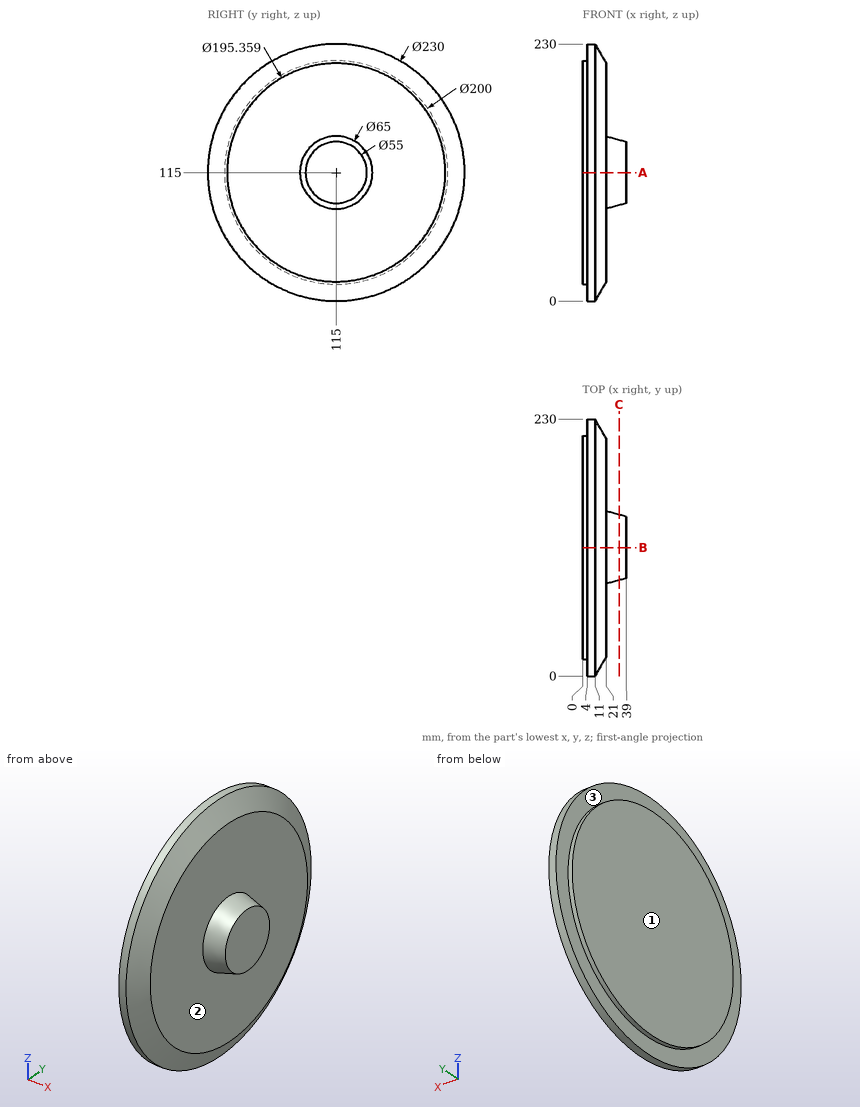
Geometry check sheet. Reference: drawing and pictorial views, mm from the part's lowest x, y, z. A direction names the side the tool comes from. Give positions to 0.01 mm unless a question says otherwise; leave off trailing zeros. Order: outer loops, then holes, each group sorted by start corner. A loop starts at its lowest first (then second) coordinate and runs counter-clockwise, first axis right, second up. Notation, with made-up numbers: M -13.5,17.5 L -9.5,17.5 A8 cw -9.5,25.5 Z; hole C 20,17.5 d5. An arc over 180 degrees is marked long. Answer in a Markdown table with one row per item. Add a question column.
Item 1: Tool access check on the marked faces 1, 2 and 3. Record the directions out of +Z, -Z, +X, -X, +Y, -Y that give a thin tool (end or side, any length) a straight path to the whole face; none if there is none.
Item 2: Section check C-C, the plane x = 32.5. Enter the section's corners in (y, z).
Item 3: Gauge pin test, flat ends, axial feed: pin 1 (2 mm diameter, centred on x = 4.5, z = 190.5, fed in from -Y); pin 2 (4 mm diameter, centred on x = 21, z = 113, fed in from -Y); pin 3 (6 mm diameter, centred on x = 5.5, y = 44, fed in from -Z). Record the tip position at first contact, or that the pin passes through.
Item 4: Section check A-A, the plane z = 115. Enter the section's corners in (x, y), and give its area (3 significant figures).
Item 5: Scan lines: probe 1 along X at (y, z) = (169, 55); probe 2 along Z at (x, y) = (34.5, 137); probe 3 along Y at (x, z) = (12, 163). Record each from-to range of solid material in increasing order. Write a range as from..to.
Filled sheet:
| question | item | result |
|---|---|---|
| 1 | face 1 | +Z, -Z, -X, +Y, -Y |
| 1 | face 2 | +X |
| 1 | face 3 | -X |
| 2 | outline | C 115,115 d58.61 |
| 3 | pin 1 | stops at y = 27.39 |
| 3 | pin 2 | stops at y = 13.88 |
| 3 | pin 3 | stops at z = 22.26 |
| 4 | outline | M 0,15 L 4,15 L 4,0 L 11,0 L 21,17.32 L 21,82.5 L 39,87.5 L 39,142.5 L 21,147.5 L 21,212.68 L 11,230 L 4,230 L 4,215 L 0,215 Z |
| 4 | area | 5,620 mm^2 |
| 5 | probe 1 | x = 0..21 |
| 5 | probe 2 | z = 96.49..133.51 |
| 5 | probe 3 | y = 12.41..217.59 |
